Build history of the part. All positions in model axes, mm. Round coordinates to 2 decimals unless told otherwise and drop trailing zeros. Write each loop counter-clockwise with the first axis right and the second up, starting at its lowest first coordinate (ties: lowest second). Pieces come first, ordered by that corner, then holes. Notation, with made-up numbers: (54.5, 86.25) -> (59.5, 86.25) arc R13 ccw to (59.5, 108.25) -> close; hole circle Ø4 at (-29.75, 51.25). An arc over 180 degrees is marked (long way). Answer as CSV lines item,"result".
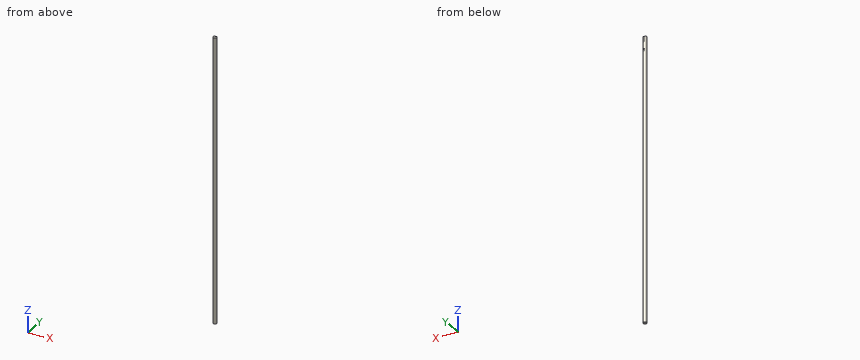
from build123d import *

# Parameters (mm, degrees)
SKETCH_1_R               = 7.5
EXTRUDE_1_DEPTH          = 1130
CUT_EXTRUDE_START        = -20
CUT_EXTRUDE_1_DEPTH      = 20
CUT_EXTRUDE_2_REACH      = 1132.089
CUT_EXTRUDE_2_END_RADIUS = 7.5
CUT_EXTRUDE_3_DEPTH      = 17


with BuildPart() as part:
    # 草图1 → 凸台-拉伸1 (new body)
    with BuildSketch(Plane.XY):
        Circle(SKETCH_1_R)
    extrude(amount=EXTRUDE_1_DEPTH)

    # 草图2 → 切除-拉伸1 (cut)
    with BuildSketch(Plane.XY.offset(1130).offset(CUT_EXTRUDE_START)):
        with BuildLine():
            Line((-2.5, 7.071067812), (-2.5, 4.5))
            Line((-2.5, 4.5), (2.5, 4.5))
            Line((2.5, 4.5), (2.5, 7.071067812))
            ThreePointArc((2.5, 7.071067812), (0, 7.5), (-2.5, 7.071067812))
        make_face()
    extrude(amount=CUT_EXTRUDE_1_DEPTH, mode=Mode.SUBTRACT)

    # 切除-拉伸2: up to this cylinder (the profile starts inside it)
    cut_extrude_2_end = Plane(origin=(0, 0, 1108.938967), z_dir=(0, 0, -1)) * Cylinder(CUT_EXTRUDE_2_END_RADIUS, 2280.178, mode=Mode.PRIVATE)
    # 草图3 → 切除-拉伸2 (cut, up to the surface)
    with BuildSketch(Plane(origin=(0, 4.5, 0), x_dir=(1, 0, 0), z_dir=(0, 1, 0)), mode=Mode.PRIVATE) as cut_extrude_2_sk1:
        with BuildLine():
            Line((-2.5, -1110), (2.5, -1110))
            ThreePointArc((2.5, -1110), (0, -1107.5), (-2.5, -1110))
        make_face()
    cut_extrude_2_tool1 = extrude(cut_extrude_2_sk1.sketch, amount=CUT_EXTRUDE_2_REACH, mode=Mode.PRIVATE) & cut_extrude_2_end
    add(cut_extrude_2_tool1.solids().sort_by_distance((0, 4.5, 1108.938967))[0], mode=Mode.SUBTRACT)

    # 草图5 → 切除-拉伸3 (cut)
    with BuildSketch(Plane(origin=(0, 4.5, 0), x_dir=(1, 0, 0), z_dir=(0, 1, 0))):
        with BuildLine():
            Line((-2.5, -1079.079030824), (-2.5, -1074.079030824))
            ThreePointArc((-2.5, -1074.079030824), (0, -1071.579030824), (2.5, -1074.079030824))
            Line((2.5, -1074.079030824), (2.5, -1079.079030824))
            ThreePointArc((2.5, -1079.079030824), (0, -1081.579030824), (-2.5, -1079.079030824))
        make_face()
    extrude(amount=CUT_EXTRUDE_3_DEPTH, mode=Mode.SUBTRACT)


solid = part.part
1. Drop flat-ended pins along their axis: pin 1 Ø0.8 at (y, z) = (6.5, 1118) entering from +X; pin 2 Ø2 at (y, z) = (5.5, 1076) entering from -X; pin 3 Ø5.5 at (x, z) = (0, 1114) entering from +Y. Give the stop position or say it passes through.
Results found:
pin 1,"stops at x = 4.36"
pin 2,"stops at x = -6"
pin 3,"stops at y = 7.07"
2. Cut at A-A, the plane z = 370.5. Write the cut outline in (x, y).
Results found:
outline,"circle Ø15 at (0, 0)"
3. Cut at B-B, the plane y = -3.75. Write the cut outline in (x, z), then the cut area to 3 significant figures.
Results found:
outline,"(-6.5, 0) -> (6.5, 0) -> (6.5, 1130) -> (-6.5, 1130) -> close"
area,"14,700 mm2"
4. Probe line 1 along Y through (x, z) = (1.25, 617); line 2 along X through (y, z) = (-0.5, 957); line 3 along Z through (x, y) = (-0.25, 6.25). List the from-to ranges inside material, lowest first.
Results found:
line 1,"y = -7.4 to 7.4"
line 2,"x = -7.48 to 7.48"
line 3,"z = 0 to 1071.59, 1081.57 to 1107.51"
